```python
from build123d import *

# Parameters (mm, degrees)
EXTRUDE_393_DEPTH = 7.5
FILLET_1265_R     = 0.6


with BuildPart() as part:
    # 草图1 → Extrude 393 (new body)
    with BuildSketch(Plane(origin=(0, 0, 0), x_dir=(0, 0, -1), z_dir=(1, 0, 0))):
        Polygon((9, 5.196152423), (9, -5.196152423), (0, -10.392304845), (-9, -5.196152423), (-9, 5.196152423), (0, 10.392304845), align=None)
    extrude(amount=EXTRUDE_393_DEPTH)

    # 草图2 → 凸台-旋转1 (revolve)
    with BuildSketch(Plane.XY, mode=Mode.PRIVATE) as revolve_1_sk:
        Polygon((0, 0), (42.5, 0), (42.5, 4.4845), (42.5, 6), (0, 6), align=None)
    revolve(revolve_1_sk.sketch.rotate(Axis((0, 0, 0), (1, 0, 0)), 90), axis=Axis((0, 0, 0), (1, 0, 0)))

    # 草图3 → 切除-旋转1 (revolve, cut)
    with BuildSketch(Plane.XY):
        Polygon((0, 9), (3.690598923, 15.392304845), (3.690598923, 20.392304845), (-10, 20.392304845), (-10, 9), align=None)
    revolve(axis=Axis((0, 0, 0), (1, 0, 0)), mode=Mode.SUBTRACT)

    # 草图4 → 切除-旋转3 (revolve, cut)
    with BuildSketch(Plane.XY, mode=Mode.PRIVATE) as cut_revolve_3_sk:
        Polygon((7.5, 8.315), (6.9, 8.661410162), (6.9, 10.392304845), (7.5, 10.392304845), align=None)
    revolve(cut_revolve_3_sk.sketch.rotate(Axis((0, 0, 0), (1, 0, 0)), 90), axis=Axis((0, 0, 0), (1, 0, 0)), mode=Mode.SUBTRACT)

    # Fillet 1265
    fillet_1265_edges = [part.edges().sort_by_distance(p)[0] for p in [
        (7.5, 0, -6),
    ]]
    fillet(fillet_1265_edges, radius=FILLET_1265_R)

    # 草图6 → 切除-旋转4 (revolve, cut)
    with BuildSketch(Plane.XY, mode=Mode.PRIVATE) as cut_revolve_4_sk:
        Polygon((41.625, 6), (43.375, 6), (42.5, 4.484455543), align=None)
    revolve(cut_revolve_4_sk.sketch.rotate(Axis((0, 0, 0), (1, 0, 0)), 90), axis=Axis((0, 0, 0), (1, 0, 0)), mode=Mode.SUBTRACT)


solid = part.part
```
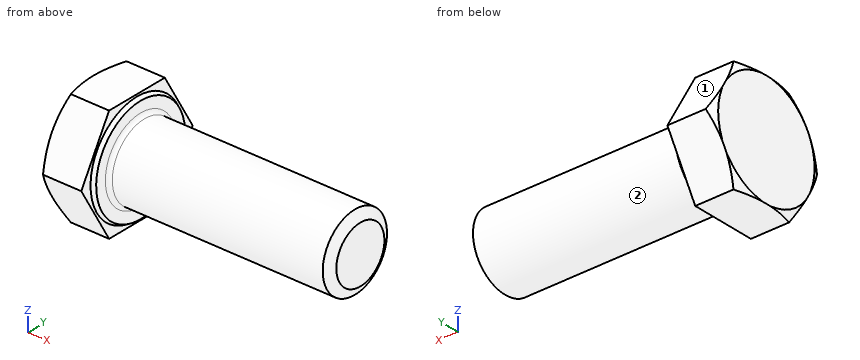
Geometry: final body of the model. Coordinates: model frame, mm. Face numbers are marked on the shaded views. A direction names the side the tool comes from. Coordinates: 2 decimals unless noted, no trailing zeros. Loops run counter-clockwise (first coordinate to the right, second up) from the corner with the lowest first, then second, coordinate; pieces in that order, holes last. Notation, with made-up numbers: (74.5, -8) -> (96.5, -8) arc R20 cw to (96.5, 23) -> close; hole circle Ø11 at (-25.75, -14.5). An arc over 180 degrees is marked (long way). Use a Markdown table: item, result. Add a question column.
(1) Pin query (flat end, axial travel): pin 1 Ø2 at (x, z) = (35, 1) entering from -Y; pin 2 Ø5 at (x, y) = (36, 4) entering from -Z; pin 3 Ø10 at (x, y) = (17, 8) entering from +Z. Return the tip coordinate at first contact, or that it passes through.
(2) Line query: line 1 along Y through (x, z) = (37, 0.25); line 2 along X through (y, z) = (-8, 3.75); line 3 along X through (y, z) = (-4.75, 5). Output: solid intervals per line, ascending.
(3) Access query for the marked faces 1 and 2. Directions: +Z, -Z, +X, -X, +Y, -Y. A direction counts if a zero-diameter tool reaches every point of the face in a straight line with its end or side. Return the directions, or none.
(4) Section query A-A, the plane x = 5.5. Return loops of the section in (y, z).
(5) Section query B-B, the plane x = 18. Return loops of the section in (y, z).
Answer:
| question | item | result |
|---|---|---|
| 1 | pin 1 | stops at y = -6 |
| 1 | pin 2 | stops at z = -5.81 |
| 1 | pin 3 | stops at z = 5.2 |
| 2 | line 1 | y = -5.99 to 5.99 |
| 2 | line 2 | x = 0 to 6.9 |
| 2 | line 3 | x = 0 to 7.5 |
| 3 | face 1 | +Z, +X, -X, +Y |
| 3 | face 2 | +X |
| 4 | outline | (-10.39, 0) -> (-5.2, -9) -> (5.2, -9) -> (10.39, 0) -> (5.2, 9) -> (-5.2, 9) -> close |
| 5 | outline | circle Ø12 at (0, 0) |
